Can you work these out from the drawing? Everything is in mm from the part's minimum corner. A direction names the side the tool comes from. Round coordinates to 2 decimals unless told otherwise and drop trailing zeros. Write each loop counter-clockwise with the first axis right and the second up, starting at its lowest first coordinate (ties: lowest second). Pieces come first, ordered by that corner, then holes. Notation, with made-up numbers: (23, 89) -> (36, 89) arc R21 ccw to (36, 97) -> close; hole circle Ø9 at (48.5, 89.25). An arc over 180 degrees is marked (long way). Write item = value, one per line. Start each with the question number.
1) If I drill on line 1 (Y direction, x = 10, z = 46); line 2 (X direction, y = 49, z = 44.5); line 3 (Z direction, x = 98.5, y = 48), over which ranges is the centre line in solid material (lowest first)?
2) Imagine slicing it at B-B, the plane y = 10. Please give me the cut outline in (x, z), then the cut area to 3 significant figures.
3) I'm going to push flat-ended pins straight in: pin 1 (1.5 mm diameter, centred on x = 87.5, z = 17.5, fed in from -Y); pin 2 (10 mm diameter, centred on x = 41, y = 52, fed in from -Z); pin 3 (5 mm diameter, centred on x = 22.5, y = 22, fed in from -Z). Where does each tip first touch, or does it pass through?
4) Imagine slicing it at A-A, the plane z = 47. Please give me the cut outline in (x, y), then the cut area to 3 significant figures.
5) For the marked faces 1, 2 and 3, which set-ups out of +Z, -Z, +X, -X, +Y, -Y let a thin tool reach every point of the face, with its end or its side?
6) Imagine slicing it at C-C, the plane x = 10. Please give me the cut outline in (y, z).
7) Imagine slicing it at D-D, the plane y = 16.5. Please give me the cut outline in (x, z), then the cut area to 3 significant figures.
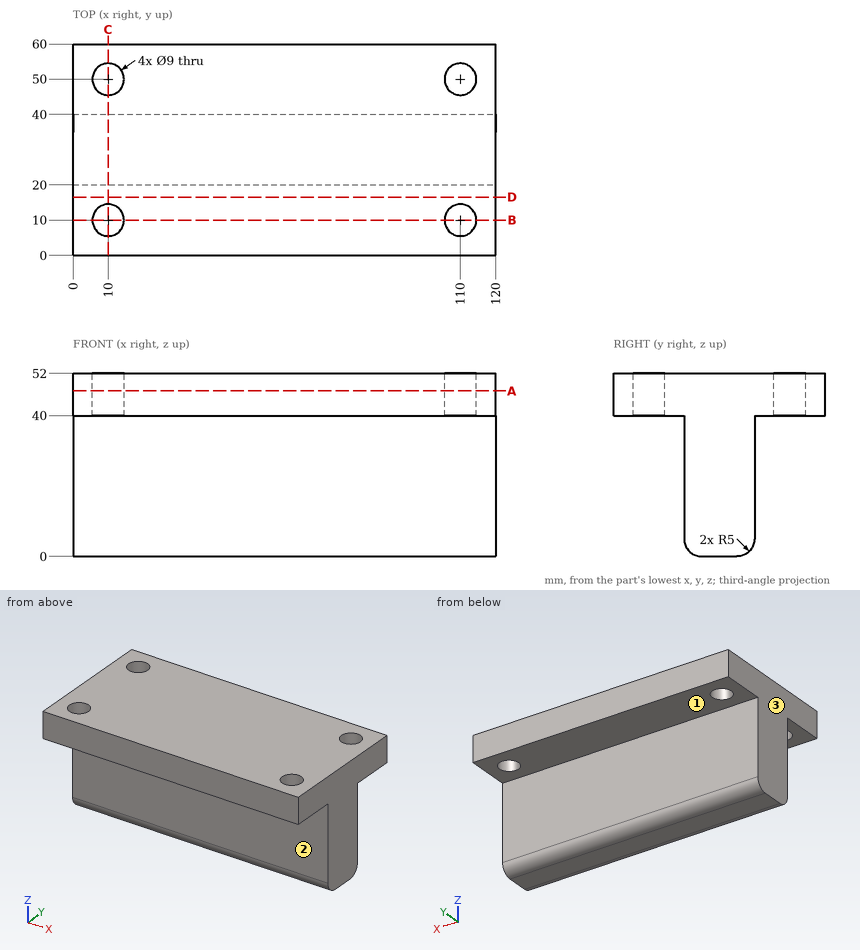
Reported:
q1.line_1 = 0 to 5.5, 14.5 to 45.5, 54.5 to 60
q1.line_2 = 0 to 5.61, 14.39 to 105.61, 114.39 to 120
q1.line_3 = 40 to 52
q2.outline = (0, 40) -> (5.5, 40) -> (5.5, 52) -> (0, 52) -> close; (14.5, 40) -> (105.5, 40) -> (105.5, 52) -> (14.5, 52) -> close; (114.5, 40) -> (120, 40) -> (120, 52) -> (114.5, 52) -> close
q2.area = 1,220 mm²
q3.pin_1 = 20
q3.pin_2 = 40
q3.pin_3 = 0.03
q4.outline = (0, 0) -> (120, 0) -> (120, 60) -> (0, 60) -> close; hole circle Ø9 at (10, 10); hole circle Ø9 at (10, 50); hole circle Ø9 at (110, 10); hole circle Ø9 at (110, 50)
q4.area = 6,950 mm²
q5.face_1 = -Z, +X, -X, +Y
q5.face_2 = -Z, +X, -X, -Y
q5.face_3 = +Z, -Z, -X, +Y, -Y
q6.outline = (0, 40) -> (5.5, 40) -> (5.5, 52) -> (0, 52) -> close; (14.5, 40) -> (20, 40) -> (20, 5) arc R5 ccw to (25, 0) -> (35, 0) arc R5 ccw to (40, 5) -> (40, 40) -> (45.5, 40) -> (45.5, 52) -> (14.5, 52) -> close; (54.5, 40) -> (60, 40) -> (60, 52) -> (54.5, 52) -> close
q7.outline = (0, 40) -> (120, 40) -> (120, 52) -> (0, 52) -> close
q7.area = 1,440 mm²
